from build123d import *

# Parameters (mm, degrees)
SKETCH_1_R          = 22.5
SKETCH_1_R_2        = 13
EXTRUDE_1_DEPTH     = 2
SKETCH_2_R          = 40
SKETCH_2_R_2        = 13
EXTRUDE_2_DEPTH     = 4
SKETCH_3_R          = 17
SKETCH_3_R_2        = 13
EXTRUDE_3_DEPTH     = 11
CHAMFER_1_SIZE      = 0.5
FILLET_1_R          = 0.5
SKETCH_4_R          = 3
CUT_EXTRUDE_1_DEPTH = 58.888606929


with BuildPart() as part:
    # 草图1 → 拉伸1 (new body)
    with BuildSketch(Plane.XY):
        Circle(SKETCH_1_R)
        Circle(SKETCH_1_R_2, mode=Mode.SUBTRACT)
    extrude(amount=EXTRUDE_1_DEPTH)

    # 草图2 → 拉伸2 (add)
    with BuildSketch(Plane.XY.offset(2)):
        with Locations((0, 0.374383119)):
            Circle(SKETCH_2_R)
        Circle(SKETCH_2_R_2, mode=Mode.SUBTRACT)
    extrude(amount=EXTRUDE_2_DEPTH)

    # 草图3 → 拉伸3 (add)
    with BuildSketch(Plane.XY.offset(6)):
        Circle(SKETCH_3_R)
        Circle(SKETCH_3_R_2, mode=Mode.SUBTRACT)
    extrude(amount=EXTRUDE_3_DEPTH)

    # 倒角1
    chamfer_1_edges = [part.edges().sort_by_distance(p)[0] for p in [
        (-40, 0.374383119, 2),
        (-17, 0, 17),
        (-13, 0, 17),
        (-22.5, 0, 0),
        (-13, 0, 0),
        (-40, 0.374383119, 6),
    ]]
    chamfer(chamfer_1_edges, length=CHAMFER_1_SIZE)

    # 圆角1
    fillet_1_edges = [part.edges().sort_by_distance(p)[0] for p in [
        (-17, 0, 6),
    ]]
    fillet(fillet_1_edges, radius=FILLET_1_R)

    # 草图4 → 切除-拉伸1 (cut, through all)
    with BuildSketch(Plane.XY.offset(6)):
        with Locations((0, 32)):
            Circle(SKETCH_4_R)
        with Locations((-32, 0)):
            Circle(SKETCH_4_R)
        with Locations((0, -32)):
            Circle(SKETCH_4_R)
        with Locations((32, 0)):
            Circle(SKETCH_4_R)
    extrude(amount=-CUT_EXTRUDE_1_DEPTH, mode=Mode.SUBTRACT)


solid = part.part
Source: CAD feature listing. Evaluate the final solid. Frame: model axes, mm. A direction names the side the tool comes from. Give positions to 0.01 mm unless a question says otherwise; leave off trailing zeros. Order: outer loops, then holes, each group sorted by start corner. A loop starts at its lowest first (then second) coordinate and runs counter-clockwise, first axis right, second up. Notation, with made-up numbers: (20, -21.5) -> (61, -21.5) arc R23 ccw to (61, 5.5) -> close; hole circle Ø7 at (48, -35). An arc over 180 degrees is marked (long way). Write item = value, one per line.
Item 1: Section query B-B (z = 14.75). Output: boundary loops of the cut face in (x, y).
Check result:
outline = circle Ø34 at (0, 0); hole circle Ø26 at (0, 0)
Item 2: Section query A-A (x = 0). State how many separate pieces and enclosed holes the cut face has, then the cut area to 3 significant figures.
Check result:
separate_pieces = 4
enclosed_holes = 0
area = 293 mm²
Item 3: Contact query for flat-ended pins moving along their axis: pin 1 (7 mm diameter, centred on x = 32, y = 0, fed in from -Z); pin 2 (5 mm diameter, centred on x = 15.5, z = 11, fed in from +Y); pin 3 (4 mm diameter, centred on y = 12, z = 14, fed in from +X). Output: stop coordinate, or through.
Check result:
pin_1 = 2
pin_2 = 10.95
pin_3 = 13.75
Item 4: Mould query, pull axis X, two halves, no side actions, for faces 4 (the face through (-2.21, 34.03, 4.03)), 5 (the face through (29, 0, 4)), 6 (the face through (10.382, -19.961, 1.24)), 7 (the face through (-14, 0, 17)). Classes: +X half, -X half, draft (parallel to the pull), parting line (faces both ways), or undercut.
Check result:
face_4 = undercut
face_5 = undercut
face_6 = parting line
face_7 = draft
Item 5: Set-up query: faces 1 (the face through (-18, 1, 6)), 2 (the face through (21.504, 34.103, 3.979)), 3 (the face through (17, -17, 2)). Return all of +Z, -Z, +X, -X, +Y, -Y with unobstructed straight access to the full face (end or side cutting, diameter ignored); none if empty.
Check result:
face_1 = +Z
face_2 = +Z, -Z
face_3 = -Z
Item 6: Ray query, probe 1 along Y at (x, z) = (0, 4.65); probe 2 along Y at (x, z) = (0, 8); probe 3 along Z at (x, y) = (0, 27). Return the intervals inside material, ascending.
Check result:
probe_1 = -39.63 to -35, -29 to -13, 13 to 29, 35 to 40.37
probe_2 = -17 to -13, 13 to 17
probe_3 = 2 to 6
